CAD build for the part. Positions are in the model's coordinates, mm. Give positions to 0.01 mm unless a question says otherwise; leave off trailing zeros. Loops run counter-clockwise (first coordinate to the right, second up) from the corner with the lowest first, then second, coordinate; pieces in that order, holes last. Notation, with made-up numbers: (-26.5, 26) -> (22.5, 26) arc R18 cw to (22.5, 39) -> close; hole circle Ø9 at (14, 33.25). An arc over 180 degrees is marked (long way). Write each question's results on one line, items separated by ' | '. Start each with the question number.
```python
from build123d import *

# Parameters (mm, degrees)
SKETCH1_W             = 190
SKETCH1_H             = 200
BOSS_EXTRUDE1_DEPTH   = 10
SKETCH2_R             = 64
CUT_EXTRUDE1_DEPTH    = 10
SKETCH3_R             = 3.5
CUT_EXTRUDE2_DEPTH    = 10
SKETCH4_W             = 27.5
SKETCH4_H             = 200
BOSS_EXTRUDE2_DEPTH   = 10
SKETCH5_R             = 5.5
CUT_EXTRUDE3_DEPTH    = 10
SKETCH6_R             = 0.5
CUT_EXTRUDE4_DEPTH    = 10
M5_TAPPED_HOLE1_D     = 4.2
M5_TAPPED_HOLE1_DEPTH = 14
M5_TAPPED_HOLE1_TIP   = 1.2618073
FILLET1_R             = 10


with BuildPart() as part:
    # Sketch1 → Boss-Extrude1 (new body)
    with BuildSketch(Plane.XY):
        Rectangle(SKETCH1_W, SKETCH1_H)
    extrude(amount=BOSS_EXTRUDE1_DEPTH)

    # Sketch2 → Cut-Extrude1 (cut)
    with BuildSketch(Plane.XY.offset(10)):
        Circle(SKETCH2_R)
    extrude(amount=-CUT_EXTRUDE1_DEPTH, mode=Mode.SUBTRACT)

    # Sketch3 → Cut-Extrude2 (cut)
    with BuildSketch(Plane.XY.offset(10)):
        with Locations((-60.25, 38.425)):
            Circle(SKETCH3_R)
        with Locations(Location((60.25, 38.425, 0), (0, 0, 180))):
            Circle(SKETCH3_R)
        with Locations((60.25, -38.425)):
            Circle(SKETCH3_R)
        with Locations(Location((-60.25, -38.425, 0), (0, 0, 180))):
            Circle(SKETCH3_R)
    extrude(amount=-CUT_EXTRUDE2_DEPTH, mode=Mode.SUBTRACT)

    # Sketch4 → Boss-Extrude2 (add)
    with BuildSketch(Plane.XY.offset(10)):
        with Locations((108.75, 0)):
            Rectangle(SKETCH4_W, SKETCH4_H)
    extrude(amount=-BOSS_EXTRUDE2_DEPTH)

    # Sketch5 → Cut-Extrude3 (cut)
    with BuildSketch(Plane.XY.offset(10)):
        with Locations((97.5, 75)):
            Circle(SKETCH5_R)
        with Locations(Location((97.5, -75, 0), (0, 0, 180))):
            Circle(SKETCH5_R)
    extrude(amount=-CUT_EXTRUDE3_DEPTH, mode=Mode.SUBTRACT)

    # Sketch6 → Cut-Extrude4 (cut)
    with BuildSketch(Plane.XY.offset(10)):
        with Locations((-87, -92)):
            Circle(SKETCH6_R)
        with Locations(Location((-87, 92, 0), (0, 0, 180))):
            Circle(SKETCH6_R)
    extrude(amount=-CUT_EXTRUDE4_DEPTH, mode=Mode.SUBTRACT)

    # M5 Tapped Hole1
    with Locations(Plane.XY.offset(10)):
        with Locations((-87, 92), (-87, -92)):
            Hole(M5_TAPPED_HOLE1_D / 2, depth=M5_TAPPED_HOLE1_DEPTH)
            with Locations((0, 0, -(M5_TAPPED_HOLE1_DEPTH + M5_TAPPED_HOLE1_TIP / 2))):  # 118° drill point
                Cone(0, M5_TAPPED_HOLE1_D / 2, M5_TAPPED_HOLE1_TIP, mode=Mode.SUBTRACT)

    # Fillet1
    fillet1_edges = [part.edges().sort_by_distance(p)[0] for p in [
        (122.5, 100, 5),
        (122.5, -100, 5),
        (-95, -100, 5),
        (-95, 100, 5),
    ]]
    fillet(fillet1_edges, radius=FILLET1_R)


solid = part.part
```
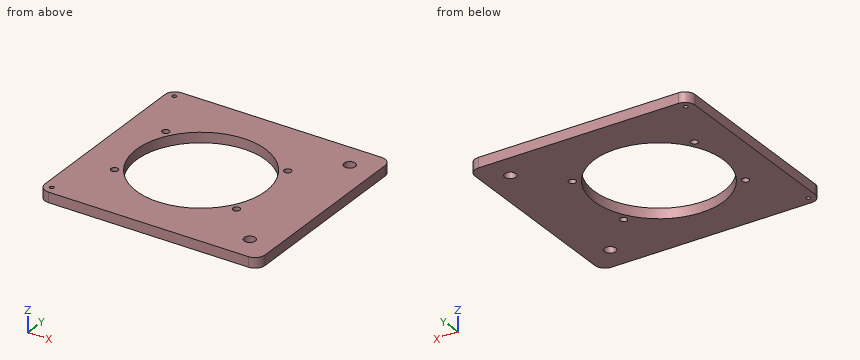
Q1. Saw through at D-D, the plane x = 60.25. List the corners of the cut face in (y, z) (3 decimals), then the cut area to 3 significant figures.
Q2. Saw through at C-C, the plane x = 0. List the corners of the cut face in (y, z), then the cut area to 3 significant figures.
Q3. Saw through at B-B, the plane y = 75. List the corners of the cut face in (x, z).
Q4. Saw through at A-A, the plane x = 97.5. List the corners of the cut face in (y, z).
Q5. Wall check: L1, parallel to Y at x = 97.5, z = 6; L2, parallel to X at y = -75, z = 3.25; L3, parallel to X at y = 77.5, z = 4.5. Give the ranges that are in metal, low to high.
Q6. Drop a flat-ended pin along its axis: pin 1 (4 mm diameter, centred on x = -87, y = -92, fed in from +Z). Give the stop position or say it passes through.
Answer block:
1) outline: (-100, 0) -> (-41.925, 0) -> (-41.925, 10) -> (-100, 10) -> close; (-34.925, 0) -> (-21.586, 0) -> (-21.586, 10) -> (-34.925, 10) -> close; (21.586, 0) -> (34.925, 0) -> (34.925, 10) -> (21.586, 10) -> close; (41.925, 0) -> (100, 0) -> (100, 10) -> (41.925, 10) -> close | area: 1,430 mm2
2) outline: (-100, 0) -> (-64, 0) -> (-64, 10) -> (-100, 10) -> close; (64, 0) -> (100, 0) -> (100, 10) -> (64, 10) -> close | area: 720 mm2
3) outline: (-95, 0) -> (92, 0) -> (92, 10) -> (-95, 10) -> close; (103, 0) -> (122.5, 0) -> (122.5, 10) -> (103, 10) -> close
4) outline: (-100, 0) -> (-80.5, 0) -> (-80.5, 10) -> (-100, 10) -> close; (-69.5, 0) -> (69.5, 0) -> (69.5, 10) -> (-69.5, 10) -> close; (80.5, 0) -> (100, 0) -> (100, 10) -> (80.5, 10) -> close
5) L1: y = -100 to -80.5, -69.5 to 69.5, 80.5 to 100 | L2: x = -95 to 92, 103 to 122.5 | L3: x = -95 to 92.6, 102.4 to 122.5
6) pin 1: passes through
